Geometry check sheet. Reference: drawing and pictorial views, mm from the part's lowest x, y, z. Give positions to 0.01 mm unless a question says otherwise; leave off trailing zeros. Order: outer loops, then holes, each group sorted by start corner. A loop starts at its lowest first (then second) coordinate and runs counter-clockwise, first axis right, second up.
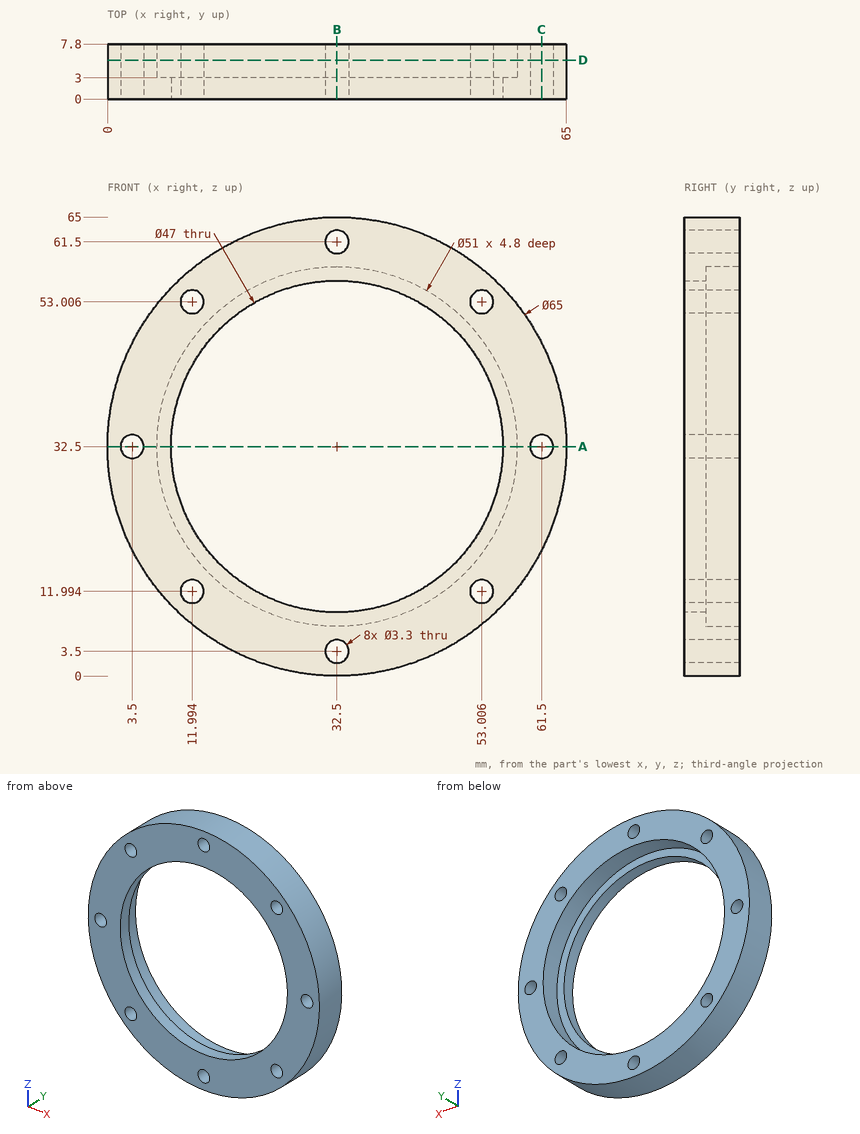
1) Section check B-B, the plane x = 32.5. Record the cut outline in (y, z).
Recorded:
outline: (0, 0) - (7.8, 0) - (7.8, 1.85) - (0, 1.85) - close; (0, 5.15) - (7.8, 5.15) - (7.8, 7) - (3, 7) - (3, 9) - (0, 9) - close; (0, 56) - (3, 56) - (3, 58) - (7.8, 58) - (7.8, 59.85) - (0, 59.85) - close; (0, 63.15) - (7.8, 63.15) - (7.8, 65) - (0, 65) - close
2) Material ranges on L1, parallel to X at y = 0.7, z = 32.5; L2, parallel to Z at x = 10.5, y = 6.25 (1 decimal); L3, parallel to Z at x = 41.5, y = 5, recorded low to high.
Recorded:
L1: x = 0 to 1.85, 5.15 to 9, 56 to 59.85, 63.15 to 65
L2: z = 8.6 to 11.3, 12.7 to 19.6, 45.4 to 52.3, 53.7 to 56.4
L3: z = 1.27 to 8.64, 56.36 to 63.73
3) Section check D-D, the plane y = 5.5. State how many separate pieces and enclosed holes the cut face has, then the cut area to 3 significant figures.
Recorded:
separate pieces: 1
enclosed holes: 9
area: 1,210 mm2
4) Section check C-C, the plane x = 61.5. Record the cut outline in (y, z), then the cut area to 3 significant figures.
Recorded:
outline: (0, 17.83) - (7.8, 17.83) - (7.8, 30.85) - (0, 30.85) - close; (0, 34.15) - (7.8, 34.15) - (7.8, 47.17) - (0, 47.17) - close
area: 203 mm2
5) Section check A-A, the plane z = 32.5. Record the cut outline in (x, y).
Recorded:
outline: (0, 0) - (1.85, 0) - (1.85, 7.8) - (0, 7.8) - close; (5.15, 0) - (9, 0) - (9, 3) - (7, 3) - (7, 7.8) - (5.15, 7.8) - close; (56, 0) - (59.85, 0) - (59.85, 7.8) - (58, 7.8) - (58, 3) - (56, 3) - close; (63.15, 0) - (65, 0) - (65, 7.8) - (63.15, 7.8) - close
6) Depth check by flat-ended pin: pin 1 Ø2 at (x, z) = (32.5, 61.5) entering from -Y; pin 2 Ø1 at (y, z) = (1.5, 26.5) entering from -X; pin 3 Ø2 at (y, z) = (2, 47) entering from +X; pin 4 Ø4.5 at (x, z) = (53.01, 11.99) entering from -Y. Enter the tip coordinate at first touch or a pass-through.
Recorded:
pin 1: passes through
pin 2: stops at x = 0.47
pin 3: stops at x = 62.06
pin 4: stops at y = 0
